The listing builds one solid part. Answer for the finished solid, in the listing's coordinates (mm). Face numbers are marked on the shaded views. A direction names the side the tool comes from. Give positions to 0.01 mm unless a question says otherwise; leave off trailing zeros. Order: outer loops, then holes, each group sorted by start corner. A loop starts at its lowest first (then second) coordinate and runs counter-clockwise, first axis right, second up. Notation, with made-up numbers: (76.5, 64.25) - (107.5, 64.25) arc R19 ccw to (107.5, 76.25) - close; hole circle Ø3 at (15.5, 57). An arc over 180 degrees is marked (long way). Answer as CSV lines item,"result". Start each with the question number.
1. Consider line 1 along Y through (x, z) = (3, 0); line 2 along X through (y, z) = (36.5, -58); line 3 along Z through (x, y) = (9, -2). Determine where each line is inside the solid, lowest interval first. Write a range as [from, to].
2. Determine the mould class of the marked faces 1, 2 and 3 for opening direction Y: +Y half, -Y half, draft (parallel to the pull), parting line (faces both ways), or undercut.
3. Which of the six approach directions +Z, -Z, +X, -X, +Y, -Y give full straight-line access (tool end or side, diameter ignored) to the marked faces 4 and 5?
4. Flat-ended cylindrical pins translate along their axes: pin 1 (19 mm diameter, centred on y = 0, z = 0, fed in from +X); pin 2 (4 mm diameter, centred on x = 11, y = -19, fed in from +Z); pin 3 (1 mm diameter, centred on x = 14, z = 59.5, fed in from -Y); pin 4 (1 mm diameter, centred on x = 28, z = 33.5, fed in from -Y). Find the tip coordinate at first contact, or state that the pin passes through.
5. Section B-B on x = 30 is taken. Give the vertices of the cut face in (y, z), and give its area (3 significant figures).
6. Section A-A on x = 9 is taken. Give the vertices of the cut face in (y, z).
from build123d import *

# Parameters (mm, degrees)
CHAMFER_1_SIZE = 1


with BuildPart() as part:
    # 草图1 → 旋转1 (revolve)
    with BuildSketch(Plane.XY, mode=Mode.PRIVATE) as revolve_1_sk:
        Polygon((0, 51), (0, 75), (7, 75), (7, 67.5), (17, 67.5), (17, 75), (26, 75), (26, 70), (32, 70), (32, 75), (40, 75), (40, 59.5), (38, 57.5), (38, 35), (40, 33), (40, 16), (13, 16), (13, 51), align=None)
    revolve(revolve_1_sk.sketch.rotate(Axis((0, 0, 0), (1, 0, 0)), 90), axis=Axis((0, 0, 0), (1, 0, 0)))

    # 倒角1
    chamfer_1_edges = [part.edges().sort_by_distance(p)[0] for p in [
        (40, 0, -75),
        (32, 0, -75),
        (26, 0, -75),
        (17, 0, -75),
        (7, 0, -75),
        (0, 0, -75),
    ]]
    chamfer(chamfer_1_edges, length=CHAMFER_1_SIZE)


solid = part.part
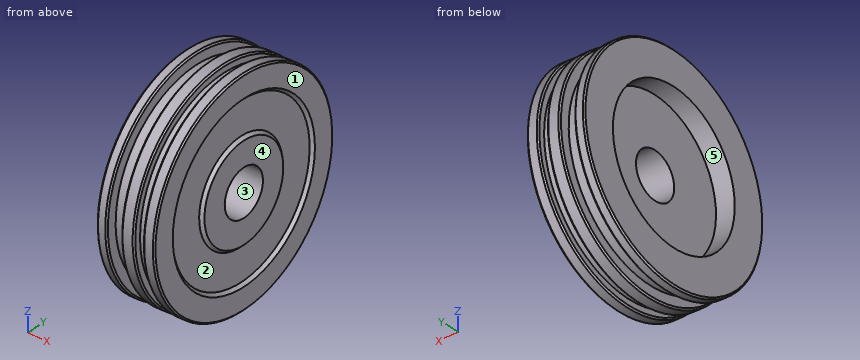
Checks:
1,line 1,"y = [-75, -51], [51, 75]"
1,line 2,"x = [0, 7], [17, 40]"
1,line 3,"z = [-67.47, -50.96], [50.96, 67.47]"
2,face 1,"draft"
2,face 2,"undercut"
2,face 3,"undercut"
3,face 4,"+Z, -Z, +X, +Y, -Y"
3,face 5,"-X"
4,pin 1,"passes through"
4,pin 2,"stops at z = 65.32"
4,pin 3,"stops at y = -32.79"
4,pin 4,"stops at y = -61.73"
5,outline,"circle Ø140 at (0, 0); hole circle Ø32 at (0, 0)"
5,area,"14,600 mm²"
6,outline,"circle Ø135 at (0, 0); hole circle Ø102 at (0, 0)"
